Input: dimensioned drawing with shaded views. Units: mm. Origin: part minimum x, y, z. Give positions to 0.01 mm unless a question says otherwise; leave off trailing zeros. Write each loop counter-clockwise with the first axis right and the second up, starting at its lowest first coordinate (ties: lowest second). Pieces come first, ordered by that corner, then holes.
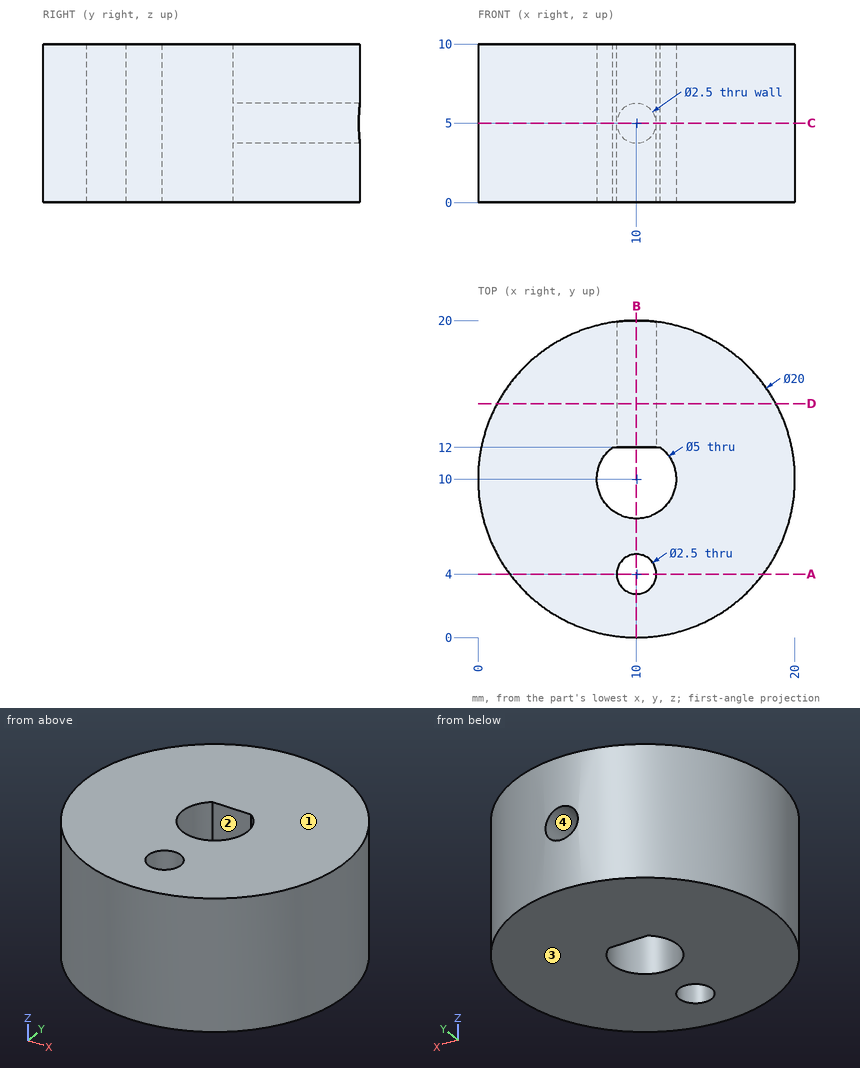
Item 1: Line query: L1, parallel to Z at x = 10, y = 14.5; L2, parallel to X at y = 10, z = 6.25; L3, parallel to X at y = 11.75, z = 6.25. Output: solid intervals per line, ascending.
Found:
L1: z = 0 to 3.75, 6.25 to 10
L2: x = 0 to 7.5, 12.5 to 20
L3: x = 0.15 to 8.21, 11.79 to 19.85
Item 2: Section C-C, the plane z = 5. Return the cut outline in (x, y).
Found:
outline: (8.5, 12) - (8.75, 12) - (8.75, 19.92) arc R10 ccw (long way) to (11.25, 19.92) - (11.25, 12) - (11.5, 12) arc R2.5 cw (long way) to start; hole circle Ø2.5 at (10, 4)
Item 3: Section A-A, the plane y = 4. Return the cut outline in (x, z), plus the area to 3 significant figures.
Found:
outline: (2, 0) - (8.75, 0) - (8.75, 10) - (2, 10) - close; (11.25, 0) - (18, 0) - (18, 10) - (11.25, 10) - close
area: 135 mm2
Item 4: Pull-direction query (Z, two-part tool) for the marked faces 1, 2, 3 and 4; classes: +Z half, -Z half, draft (parallel to the pull), parting line (faces both ways), or undercut.
Found:
face 1: +Z half
face 2: draft
face 3: -Z half
face 4: undercut
Item 5: Section B-B, the plane x = 10. Return the cut outline in (y, z), plus the area to 3 significant figures.
Found:
outline: (0, 0) - (2.75, 0) - (2.75, 10) - (0, 10) - close; (5.25, 0) - (7.5, 0) - (7.5, 10) - (5.25, 10) - close; (12, 0) - (20, 0) - (20, 3.75) - (12, 3.75) - close; (12, 6.25) - (20, 6.25) - (20, 10) - (12, 10) - close
area: 110 mm2
Item 6: Pin query (flat end, axial travel): pin 1 Ø1.5 at (x, z) = (3, 9) entering from +Y; pin 2 Ø4 at (y, z) = (2, 4.5) entering from -X; pin 3 Ø1.5 at (y, z) = (2.5, 1) entering from -X. Return the tip coordinate at first contact, or that it passes through.
Found:
pin 1: stops at y = 17.81
pin 2: stops at x = 2
pin 3: stops at x = 2.62
Item 7: Section D-D, the plane y = 14.75. Return the cut outline in (x, z), plus the area to 3 significant figures.
Found:
outline: (1.2, 0) - (18.8, 0) - (18.8, 10) - (1.2, 10) - close; hole circle Ø2.5 at (10, 5)
area: 171 mm2
